Work out the finished part from the listing and answer in its coordinate system (mm). A direction names the side the tool comes from. Round coordinates to 2 decimals unless told otherwise and drop trailing zeros. Loops run counter-clockwise (first coordinate to the right, second up) from the corner with the lowest first, then second, coordinate; pieces in that order, holes last.
```python
from build123d import *

# Parameters (mm, degrees)
SKETCH_1_W                   = 125
SKETCH_1_H                   = 80
EXTRUDE_1_DEPTH              = 7.5
HOLE_WIZARD_M8_1_D           = 9
HOLE_WIZARD_M8_1_CBORE_D     = 15
HOLE_WIZARD_M8_1_CBORE_DEPTH = 8.6
HOLE_WIZARD_M6_1_D           = 6.6
HOLE_WIZARD_M6_1_CBORE_D     = 11
HOLE_WIZARD_M6_1_CBORE_DEPTH = 6.4
CHAMFER_1_SIZE               = 2


with BuildPart() as part:
    # 草图1 → 凸台-拉伸1 (new, symmetric)
    with BuildSketch(Plane.XY):
        Rectangle(SKETCH_1_W, SKETCH_1_H)
    extrude(amount=EXTRUDE_1_DEPTH, both=True)

    # M8 六角凹头螺钉的柱形沉头孔1 (through all)
    with Locations(Plane.XY.offset(7.5)):
        with Locations((-52.5, 30), (-52.5, -30), (52.5, -30), (52.5, 30)):
            CounterBoreHole(HOLE_WIZARD_M8_1_D / 2, HOLE_WIZARD_M8_1_CBORE_D / 2, HOLE_WIZARD_M8_1_CBORE_DEPTH)

    # M6 六角凹头螺钉的柱形沉头孔1 (through all)
    with Locations(Plane(origin=(0, 0, -7.5), x_dir=(-1, 0, 0), z_dir=(0, 0, -1))):
        with Locations((-20, -20), (-20, 20), (20, -20), (20, 20)):
            CounterBoreHole(HOLE_WIZARD_M6_1_D / 2, HOLE_WIZARD_M6_1_CBORE_D / 2, HOLE_WIZARD_M6_1_CBORE_DEPTH)

    # 倒角1
    chamfer_1_edges = [part.edges().sort_by_distance(p)[0] for p in [
        (62.5, -40, 0),
        (-62.5, -40, 0),
        (-62.5, 40, 0),
        (62.5, 40, 0),
    ]]
    chamfer(chamfer_1_edges, length=CHAMFER_1_SIZE)


solid = part.part
```
1. Consider probe 1 along Y at (x, z) = (-52.5, -5.75); probe 2 along Y at (x, z) = (-20, -2.75); probe 3 along X at (y, z) = (29, 5.25). Determine where each line is inside the solid, lowest interval first.
Answer key:
probe 1: y = -40 to -34.5, -25.5 to 25.5, 34.5 to 40
probe 2: y = -40 to -25.5, -14.5 to 14.5, 25.5 to 40
probe 3: x = -62.5 to -59.93, -45.07 to 45.07, 59.93 to 62.5
2. Given pin 1 (12 mm diameter, centred on x = -51.5, y = -28, fed in from +Z); pin 2 (14.5 mm diameter, centred on x = -52.5, y = -30, fed in from +Z); pin 3 (5.5 mm diameter, centred on x = -20, y = -20, fed in from +Z), each flat-ended and moving along its own axis, determine where each tip first touches the part or whether it passes through.
Answer key:
pin 1: stops at z = 7.5
pin 2: stops at z = -1.1
pin 3: passes through
3. Determine the mould class of faces 1 (the face through (17.043, 24.638, -4.345)), 2 (the face through (-1, 40, 0)) for opening direction X: +X half, -X half, draft (parallel to the pull), parting line (faces both ways), or undercut.
Answer key:
face 1: undercut
face 2: draft
4. Which of the six approach directions +Z, -Z, +X, -X, +Y, -Y give full straight-line access (tool end or side, diameter ignored) to faces 3 (the face through (-54.58, 26.01, -4.34)), 4 (the face through (52, -35, -1.1)), 5 (the face through (-20, -24, -1.1))?
Answer key:
face 3: +Z, -Z
face 4: +Z
face 5: -Z
5. Find section C-C (z = 6.25). Give the number of separate pieces and of enclosed holes in the cut face, then the cut area to 3 significant figures.
Answer key:
separate pieces: 1
enclosed holes: 8
area: 9,150 mm2
6. Find section A-A (x = -20). Write down the section's boundary in (y, z), then the cut area to 3 significant figures.
Answer key:
outline: (-40, -7.5) - (-25.5, -7.5) - (-25.5, -1.1) - (-23.3, -1.1) - (-23.3, 7.5) - (-40, 7.5) - close; (-16.7, -1.1) - (-14.5, -1.1) - (-14.5, -7.5) - (14.5, -7.5) - (14.5, -1.1) - (16.7, -1.1) - (16.7, 7.5) - (-16.7, 7.5) - close; (23.3, -1.1) - (25.5, -1.1) - (25.5, -7.5) - (40, -7.5) - (40, 7.5) - (23.3, 7.5) - close
area: 946 mm2
7. Find section B-B (y = 20). Write down the section's boundary in (x, z).
Answer key:
outline: (-62.5, -7.5) - (-25.5, -7.5) - (-25.5, -1.1) - (-23.3, -1.1) - (-23.3, 7.5) - (-62.5, 7.5) - close; (-16.7, -1.1) - (-14.5, -1.1) - (-14.5, -7.5) - (14.5, -7.5) - (14.5, -1.1) - (16.7, -1.1) - (16.7, 7.5) - (-16.7, 7.5) - close; (23.3, -1.1) - (25.5, -1.1) - (25.5, -7.5) - (62.5, -7.5) - (62.5, 7.5) - (23.3, 7.5) - close
